For this review, take the finished solid that the model builds, in its own axes (mm). A direction names the side the tool comes from. Coordinates: 2 decimals unless noted, no trailing zeros. Loops run counter-clockwise (first coordinate to the right, second up) from the corner with the lowest first, then second, coordinate; pieces in that order, holes last. Notation, with made-up numbers: M 11,79 L 31,79 A13 ccw 31,88 Z; hole C -22,83.5 d5. An arc over 180 degrees is marked long. Put each result on its own line as item: value.
```python
from build123d import *

# Parameters (mm, degrees)
SKETCH1_W                                            = 80
SKETCH1_H                                            = 15
EXTRUDE_THIN1_DEPTH                                  = 16
HOLE_SIZE_BY_SOCKET_HEAD_CAP_SCREW_TYPE1_D           = 4.5
HOLE_SIZE_BY_SOCKET_HEAD_CAP_SCREW_TYPE1_CBORE_D     = 8
HOLE_SIZE_BY_SOCKET_HEAD_CAP_SCREW_TYPE1_CBORE_DEPTH = 4.6
SKETCH4_R                                            = 5
CUT_EXTRUDE1_DEPTH                                   = 83.95179323
M5_TAPPED_HOLE2_D                                    = 4.2
M5_TAPPED_HOLE2_DEPTH                                = 10
M5_TAPPED_HOLE2_TIP                                  = 1.2618073
M5_TAPPED_HOLE1_D                                    = 4.2
M5_TAPPED_HOLE1_DEPTH                                = 10
M5_TAPPED_HOLE1_TIP                                  = 1.2618073
CHAMFER1_SIZE                                        = 0.5


with BuildPart() as part:
    # Sketch1 → Extrude-Thin1 (new, symmetric)
    with BuildSketch(Plane.XY):
        with Locations((40, -7.5)):
            Rectangle(SKETCH1_W, SKETCH1_H)
    extrude(amount=EXTRUDE_THIN1_DEPTH, both=True)

    # Hole size by socket head cap screw type1 (through all)
    with Locations(Plane(origin=(0, -15, 0), x_dir=(-1, 0, 0), z_dir=(0, -1, 0))):
        with Locations((-68, -11), (-68, 11), (-12, -11), (-12, 11)):
            CounterBoreHole(HOLE_SIZE_BY_SOCKET_HEAD_CAP_SCREW_TYPE1_D / 2, HOLE_SIZE_BY_SOCKET_HEAD_CAP_SCREW_TYPE1_CBORE_D / 2, HOLE_SIZE_BY_SOCKET_HEAD_CAP_SCREW_TYPE1_CBORE_DEPTH)

    # Sketch4 → Cut-Extrude1 (cut, through all)
    with BuildSketch(Plane.XZ.offset(15)):
        with Locations(Location((17, 0, 0), (0, 0, 270))):
            Circle(SKETCH4_R)
        with Locations(Location((63, 0, 0), (0, 0, 270))):
            Circle(SKETCH4_R)
    extrude(amount=-CUT_EXTRUDE1_DEPTH, mode=Mode.SUBTRACT)

    # M5 Tapped Hole2
    with Locations(Plane(origin=(80, 0, 0), x_dir=(0, 0, -1), z_dir=(1, 0, 0))):
        with Locations((-7.5, -7.5), (7.5, -7.5)):
            Hole(M5_TAPPED_HOLE2_D / 2, depth=M5_TAPPED_HOLE2_DEPTH)
            with Locations((0, 0, -(M5_TAPPED_HOLE2_DEPTH + M5_TAPPED_HOLE2_TIP / 2))):  # 118° drill point
                Cone(0, M5_TAPPED_HOLE2_D / 2, M5_TAPPED_HOLE2_TIP, mode=Mode.SUBTRACT)

    # M5 Tapped Hole1
    with Locations(Plane(origin=(0, -24.315194206, 11.709083439), x_dir=(0, 0, 1), z_dir=(-1, 0, 0))):
        with Locations((-19.209083439, 16.815194206), (-4.209083439, 16.815194206)):
            Hole(M5_TAPPED_HOLE1_D / 2, depth=M5_TAPPED_HOLE1_DEPTH)
            with Locations((0, 0, -(M5_TAPPED_HOLE1_DEPTH + M5_TAPPED_HOLE1_TIP / 2))):  # 118° drill point
                Cone(0, M5_TAPPED_HOLE1_D / 2, M5_TAPPED_HOLE1_TIP, mode=Mode.SUBTRACT)

    # Chamfer1
    chamfer1_edges = [part.edges().sort_by_distance(p)[0] for p in [
        (40, 0, 16),
        (0, -7.5, 16),
        (0, -7.5, -16),
        (40, -15, 16),
        (40, 0, -16),
        (17, 0, 5),
        (17, -15, 5),
        (80, -7.5, -16),
        (63, 0, 5),
        (63, -15, 5),
        (40, -15, -16),
        (0, -15, 0),
        (0, 0, 0),
        (80, 0, 0),
        (80, -15, 0),
        (80, -7.5, 16),
    ]]
    chamfer(chamfer1_edges, length=CHAMFER1_SIZE)


solid = part.part
```
(1) Add section C-C (x = 63). Write out the cut boundary in (y, z), plus the area to 3 significant figures.
Determined:
outline: M -15,-15.5 L -14.5,-16 L -0.5,-16 L 0,-15.5 L 0,-5.5 L -0.5,-5 L -14.5,-5 L -15,-5.5 Z; M -15,5.5 L -14.5,5 L -0.5,5 L 0,5.5 L 0,15.5 L -0.5,16 L -14.5,16 L -15,15.5 Z
area: 329 mm^2
(2) Wall thickness on line 1 along X through (y, z) = (-2.75, 0); line 2 along Z through (x, y) = (5.25, -7.5); line 3 along X through (y, z) = (-7, 11): over which ranges is each line inside the solid? List them lowest first. Write a range as [from, to].
Determined:
line 1: x = [0, 12], [22, 58], [68, 80]
line 2: z = [-16, -9.6], [-5.4, 5.4], [9.6, 16]
line 3: x = [0, 9.75], [14.25, 65.75], [70.25, 80]
(3) Add section D-D (z = 0). Write out the cut boundary in (x, y), plus the area to 4 significant figures.
Determined:
outline: M 0,-14.5 L 0.5,-15 L 11.5,-15 L 12,-14.5 L 12,-0.5 L 11.5,0 L 0.5,0 L 0,-0.5 Z; M 22,-14.5 L 22.5,-15 L 57.5,-15 L 58,-14.5 L 58,-0.5 L 57.5,0 L 22.5,0 L 22,-0.5 Z; M 68,-14.5 L 68.5,-15 L 79.5,-15 L 80,-14.5 L 80,-0.5 L 79.5,0 L 68.5,0 L 68,-0.5 Z
area: 898.5 mm^2
(4) Add section B-B (z = 11). Write out the cut boundary in (x, y), plus the area to 3 significant figures.
Determined:
outline: M 0,-14.5 L 0.5,-15 L 8,-15 L 8,-10.4 L 9.75,-10.4 L 9.75,0 L 0.5,0 L 0,-0.5 Z; M 14.25,-10.4 L 16,-10.4 L 16,-15 L 64,-15 L 64,-10.4 L 65.75,-10.4 L 65.75,0 L 14.25,0 Z; M 70.25,-10.4 L 72,-10.4 L 72,-15 L 79.5,-15 L 80,-14.5 L 80,-0.5 L 79.5,0 L 70.25,0 Z
area: 1,030 mm^2
(5) Add section A-A (y = -4.5). Write out the cut boundary in (x, z).
Determined:
outline: M 0,-15.5 L 0.5,-16 L 79.5,-16 L 80,-15.5 L 80,15.5 L 79.5,16 L 0.5,16 L 0,15.5 Z; hole C 12,-11 d4.5; hole C 12,11 d4.5; hole C 17,0 d10; hole C 63,0 d10; hole C 68,-11 d4.5; hole C 68,11 d4.5
(6) Tool access review of faces 4 (the cylindrical face through (66.34, -5.13, -12.52)), 5 (the cylindrical face through (64.185, -12.732, -12.201)), 6 (the cylindrical face through (74.93, -5.418, 7.227)): name each direction out of +Z, -Z, +X, -X, +Y, -Y from which nothing blocks a thin tool from reaching the whole face with its end or side.
Determined:
face 4: +Y, -Y
face 5: -Y
face 6: +X
(7) For pin 1 (4 mm diameter, centred on y = -7.5, z = -7.5, fed in from -X); pin 2 (2.5 mm diameter, centred on x = 12.5, z = -12.5, fed in from -Y); pin 3 (3.5 mm diameter, centred on y = -7.5, z = 7.5, fed in from +X), all flat-tipped, find the tip position at first contact; note any pin that passes through.
Determined:
pin 1: stops at x = 10.06
pin 2: stops at y = -10.4
pin 3: stops at x = 69.79
(8) Draft analysis for pull direction Z (two halves, no side actions). For faces 1 (the flat face through (0, -8, 0)), 2 (the flat face through (39, -7, 16)), 3 (the cylindrical face through (67, -8, -3)), state which applies: +Z half, -Z half, draft (parallel to the pull), parting line (faces both ways), or undercut.
Determined:
face 1: draft
face 2: +Z half
face 3: undercut
